```python
from build123d import *

# Parameters (mm, degrees)
SKETCH_1_W                = 35
SKETCH_1_H                = 55
EXTRUDE_1_DEPTH           = 10
SKETCH_2_R                = 8.25
CUT_EXTRUDE_1_DEPTH       = 110
HOLE_WIZARD_M6_1_D        = 5
HOLE_WIZARD_M4_1_D        = 3.3
HOLE_WIZARD_M4_1_DEPTH    = 10.1
HOLE_WIZARD_M4_1_TIP      = 0.991420021
HOLE_WIZARD_5_0_5_1_D     = 5
HOLE_WIZARD_5_0_5_1_DEPTH = 10.1
HOLE_WIZARD_5_0_5_1_TIP   = 1.502151548
CHAMFER_1_SIZE            = 2


with BuildPart() as part:
    # 草图1 → 凸台-拉伸1 (new body)
    with BuildSketch(Plane(origin=(0, 0, 0), x_dir=(0, 0, -1), z_dir=(1, 0, 0))):
        Rectangle(SKETCH_1_W, SKETCH_1_H)
    extrude(amount=EXTRUDE_1_DEPTH)

    # 草图2 → 切除-拉伸1 (cut)
    with BuildSketch(Plane.ZY):
        with Locations((-6, 0)):
            Circle(SKETCH_2_R)
    extrude(amount=-CUT_EXTRUDE_1_DEPTH, mode=Mode.SUBTRACT)

    # M6 螺纹孔1 (through all)
    with Locations(Plane.ZY):
        with Locations((-7.5, -19)):
            hole_wizard_m6_1 = Hole(HOLE_WIZARD_M6_1_D / 2)

    # 镜向1: M6 螺纹孔1 across plane
    add(hole_wizard_m6_1.mirror(Plane.ZX), mode=Mode.SUBTRACT)

    # M4 螺纹孔1
    with Locations(Plane.XY.offset(17.5)):
        with Locations((5, 20), (5, -20)):
            Hole(HOLE_WIZARD_M4_1_D / 2, depth=HOLE_WIZARD_M4_1_DEPTH)
            with Locations((0, 0, -(HOLE_WIZARD_M4_1_DEPTH + HOLE_WIZARD_M4_1_TIP / 2))):  # 118° drill point
                Cone(0, HOLE_WIZARD_M4_1_D / 2, HOLE_WIZARD_M4_1_TIP, mode=Mode.SUBTRACT)

    # Ø5.0 (5) 直径孔1
    with Locations(Plane.XY.offset(17.5)):
        with Locations((5, 12.5), (5, -12.5)):
            Hole(HOLE_WIZARD_5_0_5_1_D / 2, depth=HOLE_WIZARD_5_0_5_1_DEPTH)
            with Locations((0, 0, -(HOLE_WIZARD_5_0_5_1_DEPTH + HOLE_WIZARD_5_0_5_1_TIP / 2))):  # 118° drill point
                Cone(0, HOLE_WIZARD_5_0_5_1_D / 2, HOLE_WIZARD_5_0_5_1_TIP, mode=Mode.SUBTRACT)

    # 倒角1
    chamfer_1_edges = [part.edges().sort_by_distance(p)[0] for p in [
        (5, -27.5, -17.5),
        (5, 27.5, -17.5),
    ]]
    chamfer(chamfer_1_edges, length=CHAMFER_1_SIZE)


solid = part.part
```
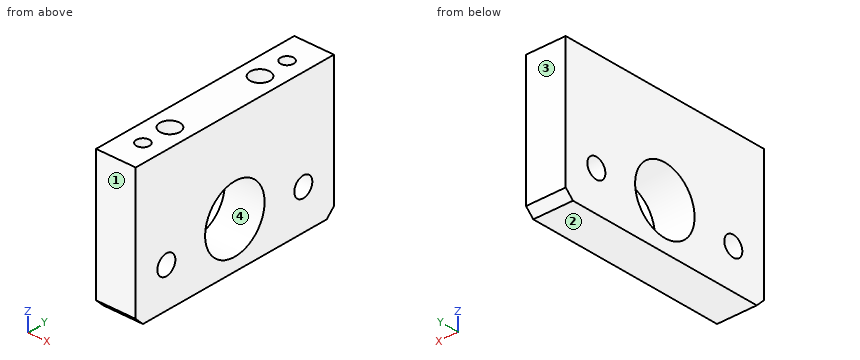
Geometry: final body of the model. Coordinates: model frame, mm. Face numbers are marked on the shaded views. Give positions to 0.01 mm unless a question says otherwise; leave off trailing zeros. Loops run counter-clockwise (first coordinate to the right, second up) from the corner with the lowest first, then second, coordinate; pieces in that order, holes last. Notation, with made-up numbers: (53.5, -2.5) -> (68.5, -2.5) arc R15 cw to (68.5, 26.5) -> close; hole circle Ø9 at (-36, 8.25). An arc over 180 degrees is marked (long way). Return JSON: item names as keys, results as strings.
Item 1: Section B-B, the plane z = -6. Output: boundary loops of the cut face in (x, y).
Filled in:
{"outline": "(0, -27.5) -> (10, -27.5) -> (10, -21) -> (0, -21) -> close; (0, -17) -> (10, -17) -> (10, -8.25) -> (0, -8.25) -> close; (0, 8.25) -> (10, 8.25) -> (10, 17) -> (0, 17) -> close; (0, 21) -> (10, 21) -> (10, 27.5) -> (0, 27.5) -> close"}
Item 2: Section D-D, the plane z = -2.5. Output: boundary loops of the cut face in (x, y).
Filled in:
{"outline": "(0, -27.5) -> (10, -27.5) -> (10, -7.47) -> (0, -7.47) -> close; (0, 7.47) -> (10, 7.47) -> (10, 27.5) -> (0, 27.5) -> close"}
Item 3: Line query: line 1 (Y direction, x = 5, z = 13.5); line 2 (X direction, y = -20, z = 13.25); line 3 (Y direction, x = 8, z = -7.5). Output: solid intervals per line, ascending.
Filled in:
{"line 1": "-27.5 to -21.65, -18.35 to -15, -10 to 10, 15 to 18.35, 21.65 to 27.5", "line 2": "0 to 3.35, 6.65 to 10", "line 3": "-27.5 to -21.5, -16.5 to -8.11, 8.11 to 16.5, 21.5 to 27.5"}
Item 4: Section A-A, the plane y = 0. Output: boundary loops of the cut face in (x, z), plus the area to 3 significant figures.
Filled in:
{"outline": "(0, -17.5) -> (10, -17.5) -> (10, -14.25) -> (0, -14.25) -> close; (0, 2.25) -> (10, 2.25) -> (10, 17.5) -> (0, 17.5) -> close", "area": "185 mm^2"}
Item 5: Mould query, pull axis Y, two halves, no side actions, for the marked faces 1, 2, 3 and 4. Classes: released by +Y, released by -Y, zero draft, split by the parting line, or undercut.
Filled in:
{"face 1": "released by -Y", "face 2": "zero draft", "face 3": "released by +Y", "face 4": "undercut"}
Item 6: Section C-C, the plane z = 10.5. Output: boundary loops of the cut face in (x, y).
Filled in:
{"outline": "(0, -27.5) -> (10, -27.5) -> (10, 27.5) -> (0, 27.5) -> close; hole circle Ø5 at (5, -12.5); hole circle Ø5 at (5, 12.5); hole circle Ø3.3 at (5, -20); hole circle Ø3.3 at (5, 20)"}
